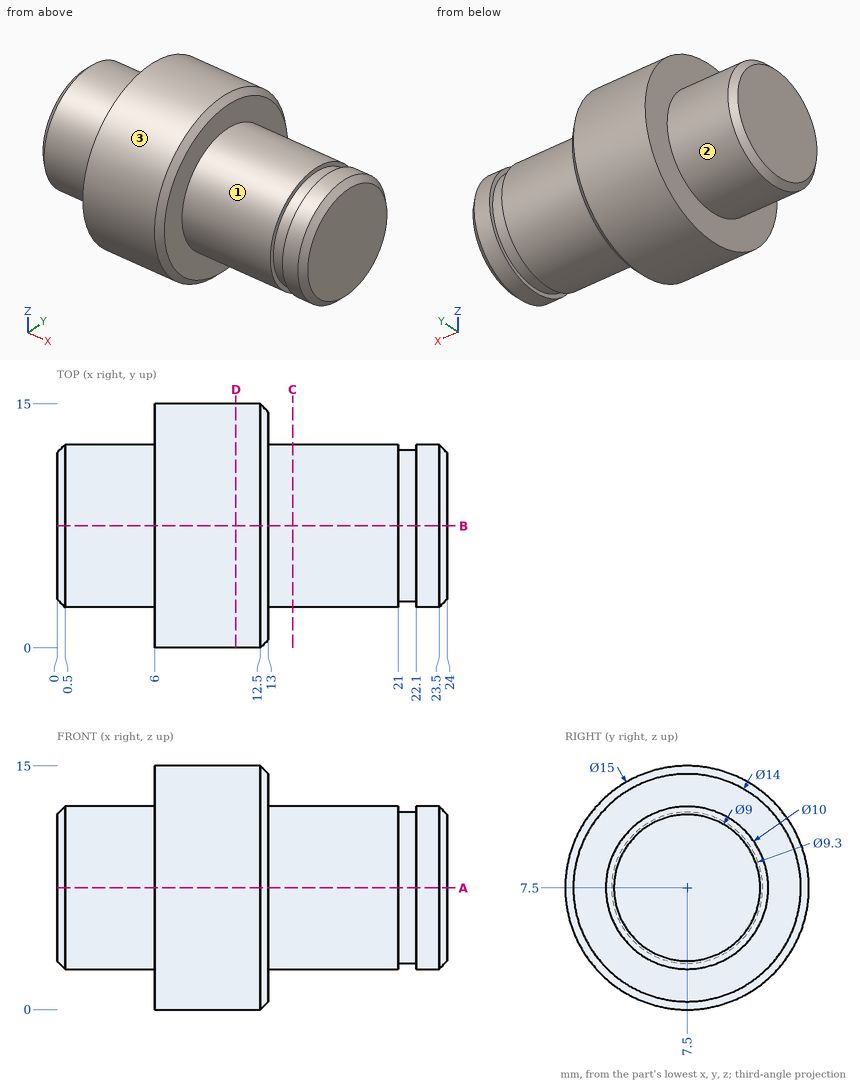
Geometry check sheet. Reference: drawing and pictorial views, mm from the part's lowest x, y, z. A direction names the side the tool comes from. Round coordinates to 2 decimals unless told otherwise and drop trailing zeros. Order: outer loops, then holes, each group sorted by start corner. A loop starts at its lowest first (then second) coordinate and runs counter-clockwise, first axis right, second up. Notation, with made-up numbers: (61, 73) -> (93, 73) arc R26 ccw to (93, 109) -> close; hole circle Ø5 at (19.25, 69). An arc over 180 degrees is marked (long way). One line per item, written item: value. Start each with the question number.
Q1. Thickness scan on line 1 (X direction, y = 2.75, z = 4.25); line 2 (Z direction, x = 17, y = 7.25); line 3 (Z direction, x = 9, y = 7.25). Record the ranges inside material, lowest first.
Q2. Cross-section at D-D (x = 11). Record the boundary of the cut face in (y, z), and give its area (3 significant figures).
Q3. Cross-section at A-A (z = 7.5). Record the boundary of the cut face in (x, y), and give its area (3 significant figures).
Q4. Gauge pin test, flat ends, axial feed: pin 1 Ø5 at (x, z) = (3, 10) entering from -Y; pin 2 Ø6 at (x, z) = (16.5, 4) entering from +Y. Record the tip position at first contact, or that the pin passes through.
Q5. Set-up check for the marked faces 1, 2 and 3: record each of +Z, -Z, +X, -X, +Y, -Y from which the full face is reachable in a straight line by a thin tool's end or side.
Q6. Cross-section at C-C (x = 14.5). Record the boundary of the cut face in (y, z).
Completed:
1. line 1: x = 6 to 13
1. line 2: z = 2.51 to 12.49
1. line 3: z = 0 to 15
2. outline: circle Ø15 at (7.5, 7.5)
2. area: 177 mm²
3. outline: (0, 3) -> (0.5, 2.5) -> (6, 2.5) -> (6, 0) -> (12.5, 0) -> (13, 0.5) -> (13, 2.5) -> (21, 2.5) -> (21, 2.85) -> (22.1, 2.85) -> (22.1, 2.5) -> (23.5, 2.5) -> (24, 3) -> (24, 12) -> (23.5, 12.5) -> (22.1, 12.5) -> (22.1, 12.15) -> (21, 12.15) -> (21, 12.5) -> (13, 12.5) -> (13, 14.5) -> (12.5, 15) -> (6, 15) -> (6, 12.5) -> (0.5, 12.5) -> (0, 12) -> close
3. area: 273 mm²
4. pin 1: stops at y = 2.5
4. pin 2: stops at y = 12.47
5. face 1: +X
5. face 2: -X
5. face 3: +X, -X
6. outline: circle Ø10 at (7.5, 7.5)
